```python
from build123d import *

# Parameters (mm, degrees)
SKETCH1_R           = 33.5
BOSS_EXTRUDE1_DEPTH = 33
SKETCH2_R           = 39.5
BOSS_EXTRUDE2_DEPTH = 20
CUT_EXTRUDE1_START  = -15
CUT_EXTRUDE1_DEPTH  = 15
SKETCH4_R           = 19.5
BOSS_EXTRUDE3_DEPTH = 3
SKETCH5_R           = 21
BOSS_EXTRUDE4_DEPTH = 67
CHAMFER1_SIZE       = 2


with BuildPart() as part:
    # Sketch1 → Boss-Extrude1 (new body)
    with BuildSketch(Plane.XY):
        Circle(SKETCH1_R)
    extrude(amount=BOSS_EXTRUDE1_DEPTH)

    # Sketch2 → Boss-Extrude2 (add)
    with BuildSketch(Plane.XY.offset(33)):
        Circle(SKETCH2_R)
    extrude(amount=BOSS_EXTRUDE2_DEPTH)

    # Sketch3 → Cut-Extrude1 (cut)
    with BuildSketch(Plane.XY.offset(53).offset(CUT_EXTRUDE1_START)):
        with BuildLine():
            Line((-22.449944321, 32.5), (22.449944321, 32.5))
            ThreePointArc((22.449944321, 32.5), (0, 39.5), (-22.449944321, 32.5))
        make_face()
        with BuildLine():
            Line((-22.449944321, -32.5), (22.449944321, -32.5))
            ThreePointArc((22.449944321, -32.5), (0, -39.5), (-22.449944321, -32.5))
        make_face()
    extrude(amount=CUT_EXTRUDE1_DEPTH, mode=Mode.SUBTRACT)

    # Sketch4 → Boss-Extrude3 (add)
    with BuildSketch(Plane.XY.offset(53)):
        Circle(SKETCH4_R)
    extrude(amount=BOSS_EXTRUDE3_DEPTH)

    # Sketch5 → Boss-Extrude4 (add)
    with BuildSketch(Plane.XY.offset(56)):
        Circle(SKETCH5_R)
    extrude(amount=BOSS_EXTRUDE4_DEPTH)

    # Chamfer1
    chamfer1_edges = [part.edges().sort_by_distance(p)[0] for p in [
        (-21, 0, 123),
    ]]
    chamfer(chamfer1_edges, length=CHAMFER1_SIZE)


solid = part.part
```
Part model, mm, in its own coordinate system. A direction names the side the tool comes from. Round coordinates to 2 decimals unless told otherwise and drop trailing zeros. Loops run counter-clockwise (first coordinate to the right, second up) from the corner with the lowest first, then second, coordinate; pieces in that order, holes last. Notation, with made-up numbers: (-8.5, 83) -> (9.5, 83) arc R17 ccw to (9.5, 109) -> close; hole circle Ø5 at (78.25, 0). An arc over 180 degrees is marked (long way). Use a Markdown table: item, result.
1) Cut at B-B, the plane x = -24. List the corners of the cut face in (y, z), and give its area (3 significant figures).
The answers:
| item | result |
|---|---|
| outline | (-31.37, 33) -> (-23.37, 33) -> (-23.37, 0) -> (23.37, 0) -> (23.37, 33) -> (31.37, 33) -> (31.37, 53) -> (-31.37, 53) -> close |
| area | 2,800 mm2 |
2) Tool access for faces 1 (the flat face through (-18, -29, 33)), 2 (the cylindrical face through (20.03, 6.31, 88.04)), 3 (the cylindrical face through (-2.539, 19.334, 54.479)), 4 (the flat face through (0, -32.5, 45)): list every direction of +Z, -Z, +X, -X, +Y, -Y with a clear straight run to the whole face (end or side of a thin tool).
The answers:
| item | result |
|---|---|
| face 1 | -Z |
| face 2 | +Z |
| face 3 | none |
| face 4 | +Z, +X, -X, -Y |
3) Cut at A-A, the plane y = 0. List the corners of the cut face in (x, z), and give its area (3 significant figures).
The answers:
| item | result |
|---|---|
| outline | (-39.5, 33) -> (-33.5, 33) -> (-33.5, 0) -> (33.5, 0) -> (33.5, 33) -> (39.5, 33) -> (39.5, 53) -> (19.5, 53) -> (19.5, 56) -> (21, 56) -> (21, 121) -> (19, 123) -> (-19, 123) -> (-21, 121) -> (-21, 56) -> (-19.5, 56) -> (-19.5, 53) -> (-39.5, 53) -> close |
| area | 6,720 mm2 |
4) Probe line 1 (Y direction, x = 9, z = 117); line 2 (Z direction, x = 10, y = 24); line 3 (Z direction, x = 34.5, y = -14.5). List the from-to ranges inside material, lowest first. Write a range as [from, to].
The answers:
| item | result |
|---|---|
| line 1 | y = [-18.97, 18.97] |
| line 2 | z = [0, 53] |
| line 3 | z = [33, 53] |
5) Cut at C-C, the plane z = 20. List the corners of the cut face in (x, y).
The answers:
| item | result |
|---|---|
| outline | circle Ø67 at (0, 0) |
6) Cut at D-D, the plane x = 0. List the corners of the cut face in (y, z), and give its area (3 significant figures).
The answers:
| item | result |
|---|---|
| outline | (-39.5, 33) -> (-33.5, 33) -> (-33.5, 0) -> (33.5, 0) -> (33.5, 33) -> (39.5, 33) -> (39.5, 38) -> (32.5, 38) -> (32.5, 53) -> (19.5, 53) -> (19.5, 56) -> (21, 56) -> (21, 121) -> (19, 123) -> (-19, 123) -> (-21, 121) -> (-21, 56) -> (-19.5, 56) -> (-19.5, 53) -> (-32.5, 53) -> (-32.5, 38) -> (-39.5, 38) -> close |
| area | 6,510 mm2 |
7) Drop flat-ended pins along their axis: pin 1 Ø16.5 at (x, z) = (-0.5, 48.5) entering from -Y; pin 2 Ø5.5 at (x, y) = (6, -35) entering from +Z; pin 3 Ø3.5 at (x, y) = (-10, 36.5) entering from +Z. Give the stop position or say it passes through.
The answers:
| item | result |
|---|---|
| pin 1 | stops at y = -32.5 |
| pin 2 | stops at z = 53 |
| pin 3 | stops at z = 38 |
